Build history of the part. All positions in model axes, mm. Face numbers are marked on the shaded views. A direction names the side the tool comes from. Round coordinates to 2 decimals unless told otherwise and drop trailing zeros. Write each loop counter-clockwise with the first axis right and the second up, starting at its lowest first coordinate (ties: lowest second). Pieces come first, ordered by that corner, then holes. Notation, with made-up numbers: M 44,80.5 L 98,80.5 A16 ccw 98,102.5 Z; hole C 69,-13 d7. An arc over 180 degrees is marked long. Use a Markdown table: item, result.
from build123d import *

# Parameters (mm, degrees)
SKETCH1_R           = 4
BOSS_EXTRUDE1_DEPTH = 3
SKETCH2_W           = 1.4
SKETCH2_H           = 9.655444372
CUT_EXTRUDE1_DEPTH  = 1.6
SKETCH3_R           = 2
BOSS_EXTRUDE2_DEPTH = 19


with BuildPart() as part:
    # Sketch1 → Boss-Extrude1 (new body)
    with BuildSketch(Plane.XY):
        Circle(SKETCH1_R)
    extrude(amount=BOSS_EXTRUDE1_DEPTH)

    # Sketch2 → Cut-Extrude1 (cut)
    with BuildSketch(Plane.XY.offset(3)):
        Rectangle(SKETCH2_W, SKETCH2_H)
    extrude(amount=-CUT_EXTRUDE1_DEPTH, mode=Mode.SUBTRACT)

    # Sketch3 → Boss-Extrude2 (add)
    with BuildSketch(Plane(origin=(0, 0, 0), x_dir=(-1, 0, 0), z_dir=(0, 0, -1))):
        Circle(SKETCH3_R)
    extrude(amount=BOSS_EXTRUDE2_DEPTH)

    # Sketch4 → Cut-Revolve5 (revolve, cut)
    with BuildSketch(Plane(origin=(0, 0, 0), x_dir=(1, 0, 0), z_dir=(0, 1, 0)), mode=Mode.PRIVATE) as cut_revolve5_sk:
        Polygon((2, 13.5), (2, 19), (0, 26.182661303), (0, 19), align=None)
    revolve(cut_revolve5_sk.sketch.rotate(Axis((0, 0, -19), (0, 0, 1)), 100.078658108), axis=Axis((0, 0, -19), (0, 0, 1)), mode=Mode.SUBTRACT)


solid = part.part
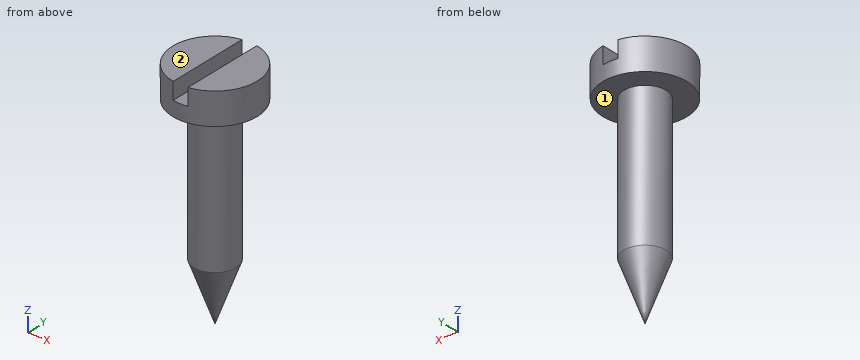
Q1. Drop flat-ended pins along their axis: P1, Ø4, axis at x = -1.5, z = -4.5, coming from the +Y side; P2, Ø0.7, axis at x = 0, y = -2, coming from the +Z side. Give the stop position or say it passes through.
Response values:
| item | result |
|---|---|
| P1 | stops at y = 2 |
| P2 | stops at z = 1.4 |
Q2. Cut at C-C on x = 3. Give the cut face in (y, z), and give its area (3 significant figures).
Response values:
| item | result |
|---|---|
| outline | M -2.65,0 L 2.65,0 L 2.65,3 L -2.65,3 Z |
| area | 15.9 mm2 |
Q3. Cut at D-D on z = -16.5. Give the cut face in (x, y), and give its area (3 significant figures).
Response values:
| item | result |
|---|---|
| outline | C 0,0 d1.82 |
| area | 2.60 mm2 |
Q4. Which spindle directions (+Z, -Z, +X, -X, +Y, -Y) get a long thin tool onto all of the face, cutting with end or side? Do the marked faces 1 and 2. Say none if no direction does.
Response values:
| item | result |
|---|---|
| face 1 | -Z |
| face 2 | +Z, +X, -X, +Y, -Y |
Q5. Cut at A-A on z = -12. Give the cut face in (x, y), and give its area (3 significant figures).
Response values:
| item | result |
|---|---|
| outline | C 0,0 d4 |
| area | 12.6 mm2 |
Q6. Drill centre lines: L1, parallel to Z at x = 2, y = 0.75; L2, parallel to Z at x = -1.25, y = 1.5; L3, parallel to X at y = 0.75, z = -12.5. Where is each one in solid material? Low to high.
Response values:
| item | result |
|---|---|
| L1 | z = 0 to 3 |
| L2 | z = -13.63 to 3 |
| L3 | x = -1.85 to 1.85 |
Q7. Cut at B-B on y = -3.25. Give the cut face in (x, z), and give its area (3 significant figures).
Response values:
| item | result |
|---|---|
| outline | M -2.33,0 L 2.33,0 L 2.33,3 L 0.7,3 L 0.7,1.4 L -0.7,1.4 L -0.7,3 L -2.33,3 Z |
| area | 11.8 mm2 |
